Job drawing, mm, ordinate dimensions from the low corner. One solid piece. Round coordinates to 2 decimals unless told otherwise and drop trailing zeros. Loops run counter-clockwise (first coordinate to the right, second up) from the corner with the lowest first, then second, coordinate; pieces in that order, holes last.
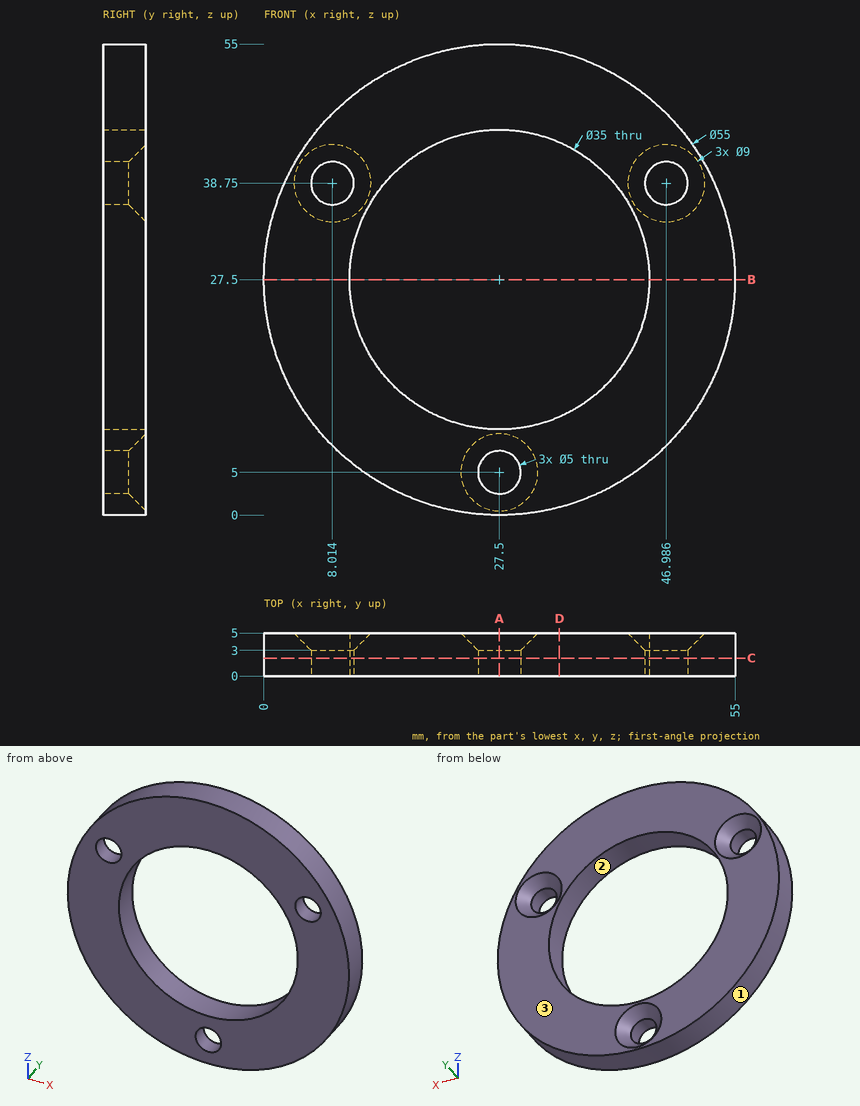
Item 1: Probe line 1 (X direction, y = 1.1, z = 38.75) (1 decimal); line 2 (X direction, y = 2.95, z = 27.5); line 3 (X direction, y = 1.2, z = 13) (1 decimal). List the from-to ranges inside material, lowest first.
Answers follow:
line 1: x = 2.4 to 5.5, 10.5 to 14.1, 40.9 to 44.5, 49.5 to 52.6
line 2: x = 0 to 10, 45 to 55
line 3: x = 4.1 to 17.7, 37.3 to 50.9
Item 2: Cut at C-C, the plane y = 2.1. State how many separate pieces and enclosed holes the cut face has, plus the area to 4 significant figures.
Answers follow:
separate pieces: 1
enclosed holes: 4
area: 1,355 mm2
Item 3: Flat gauge pins, fed straight in: P1, Ø5, axis at x = 29.5, z = 41, coming from the +Y side; P2, Ø3, axis at x = 11.5, y = 4, coming from the -Z side; P3, Ø8, axis at x = 25, z = 7.5, coming from the +Y side; P4, Ø1.5, axis at y = 3.5, z = 24, coming from the -X side. Where does each tip first touch, or does it go through?
Answers follow:
P1: passes through
P2: stops at z = 4.13
P3: stops at y = 5
P4: stops at x = 0.14
Item 4: Two-plate mould, pull along Z, no slides. Class the marked faces 1, 2 and 3: released by +Z, released by -Z, zero draft, split by the parting line, or undercut.
Answers follow:
face 1: split by the parting line
face 2: undercut
face 3: zero draft
Item 5: Cut at D-D, the plane x = 34.5. Give the cut face in (y, z) (1 decimal).
Answers follow:
outline: (0, 0.9) - (5, 0.9) - (5, 11.5) - (0, 11.5) - close; (0, 43.5) - (5, 43.5) - (5, 54.1) - (0, 54.1) - close
Item 6: Cut at B-B, the plane z = 27.5. Give the cut face in (x, y).
Answers follow:
outline: (0, 0) - (10, 0) - (10, 5) - (0, 5) - close; (45, 0) - (55, 0) - (55, 5) - (45, 5) - close
Item 7: Cut at A-A, the plane x = 27.5. Give the cut face in (y, z), plus the area to 3 significant figures.
Answers follow:
outline: (0, 0) - (5, 0) - (5, 0.5) - (3, 2.5) - (0, 2.5) - close; (0, 7.5) - (3, 7.5) - (5, 9.5) - (5, 10) - (0, 10) - close; (0, 45) - (5, 45) - (5, 55) - (0, 55) - close
area: 71.0 mm2
